```python
from build123d import *

# Parameters (mm, degrees)
SKETCH_1_W                   = 50
SKETCH_1_H                   = 120
EXTRUDE_1_DEPTH              = 6
HOLE_WIZARD_M4_1_D           = 4.5
HOLE_WIZARD_M4_1_CBORE_D     = 8
HOLE_WIZARD_M4_1_CBORE_DEPTH = 4.6
HOLE_WIZARD_M5_3_D           = 5.5
HOLE_WIZARD_M5_3_CBORE_D     = 9.5
HOLE_WIZARD_M5_3_CBORE_DEPTH = 5.7
HOLE_WIZARD_M6_1_D           = 5
HOLE_WIZARD_M6_1_DEPTH       = 15
HOLE_WIZARD_M6_1_TIP         = 1.502151548
HOLE_WIZARD_M5_1_D           = 5.5
HOLE_WIZARD_M5_1_CBORE_D     = 10
HOLE_WIZARD_M5_1_CBORE_DEPTH = 5.7
CHAMFER_1_SIZE               = 1
HOLE_WIZARD_M5_4_D           = 5.5
HOLE_WIZARD_M5_4_CBORE_D     = 10
HOLE_WIZARD_M5_4_CBORE_DEPTH = 5.7


with BuildPart() as part:
    # 草图1 → 凸台-拉伸1 (new, symmetric)
    with BuildSketch(Plane(origin=(0, 0, 0), x_dir=(1, 0, 0), z_dir=(0, 1, 0))):
        Rectangle(SKETCH_1_W, SKETCH_1_H)
    extrude(amount=EXTRUDE_1_DEPTH, both=True)

    # M4 六角圆柱头螺钉的柱形沉头孔1 (through all)
    with Locations(Plane(origin=(0, 6, 0), x_dir=(1, 0, 0), z_dir=(0, 1, 0))):
        with Locations((2, 15), (-20, 30), (2, 30), (-20, 15), (-20, -15), (2, -30), (-20, -30), (2, -15)):
            CounterBoreHole(HOLE_WIZARD_M4_1_D / 2, HOLE_WIZARD_M4_1_CBORE_D / 2, HOLE_WIZARD_M4_1_CBORE_DEPTH)

    # M5 六角圆柱头螺钉的柱形沉头孔3 (through all)
    with Locations(Plane(origin=(0, -6, 0), x_dir=(-1, 0, 0), z_dir=(0, -1, 0))):
        with Locations((16.499999999, -55), (1.500000001, -55), (1.500000001, 55), (16.499999999, 55)):
            CounterBoreHole(HOLE_WIZARD_M5_3_D / 2, HOLE_WIZARD_M5_3_CBORE_D / 2, HOLE_WIZARD_M5_3_CBORE_DEPTH)

    # M6 螺纹孔1
    with Locations(Plane(origin=(0, 6, 0), x_dir=(1, 0, 0), z_dir=(0, 1, 0))):
        with Locations((-9, 10), (-9, -10)):
            Hole(HOLE_WIZARD_M6_1_D / 2, depth=HOLE_WIZARD_M6_1_DEPTH)
            with Locations((0, 0, -(HOLE_WIZARD_M6_1_DEPTH + HOLE_WIZARD_M6_1_TIP / 2))):  # 118° drill point
                Cone(0, HOLE_WIZARD_M6_1_D / 2, HOLE_WIZARD_M6_1_TIP, mode=Mode.SUBTRACT)

    # M5 六角圆柱头螺钉的柱形沉头孔1 (through all)
    with Locations(Plane(origin=(0, 6, 0), x_dir=(1, 0, 0), z_dir=(0, 1, 0))):
        with Locations((1, 40), (1, -40), (-19, -40), (-19, 40)):
            CounterBoreHole(HOLE_WIZARD_M5_1_D / 2, HOLE_WIZARD_M5_1_CBORE_D / 2, HOLE_WIZARD_M5_1_CBORE_DEPTH)

    # 倒角1
    chamfer_1_edges = [part.edges().sort_by_distance(p)[0] for p in [
        (25, 0, 60),
        (-25, 0, 60),
        (-25, 0, -60),
        (25, 0, -60),
    ]]
    chamfer(chamfer_1_edges, length=CHAMFER_1_SIZE)

    # M5 六角圆柱头螺钉的柱形沉头孔4 (through all)
    with Locations(Plane(origin=(0, -6, 0), x_dir=(-1, 0, 0), z_dir=(0, -1, 0))):
        with Locations((-14.5, 50), (-14.5, 0), (-14.5, -50)):
            CounterBoreHole(HOLE_WIZARD_M5_4_D / 2, HOLE_WIZARD_M5_4_CBORE_D / 2, HOLE_WIZARD_M5_4_CBORE_DEPTH)


solid = part.part
```
CAD build for the part. Positions are in the model's coordinates, mm. A direction names the side the tool comes from. Coordinates: 2 decimals unless noted, no trailing zeros. Order: outer loops, then holes, each group sorted by start corner. A loop starts at its lowest first (then second) coordinate and runs counter-clockwise, first axis right, second up. Notation, with made-up numbers: M -39.75,66.5 L -20.75,66.5 A9 cw -20.75,83.5 Z; hole C 3.5,-28 d10. An arc over 180 degrees is marked long. Write each question's results on one line, items separated by ' | '. Start each with the question number.
Q1. Cut at A-A (x = 14.5). List the corners of the cut face in (y, z), then the cut area to 3 significant figures.
Q2. Which spindle directions (+Z, -Z, +X, -X, +Y, -Y) get a long thin tool onto all of the face, cutting with end or side? Do faces 1 (the flat face through (12, -0.3, -48)), 2 (the flat face through (4, 1.4, 32)), 3 (the cylindrical face through (0.79, -2.352, -31.897)). Say none if no direction does.
Q3. Pull direction Z, two halves, no side cores. Call faces 4 (the flat face through (0, 0, -60)), 5 (the flat face through (25, 0, 1)), 6 (the flat face through (-4, -0.3, 57)): +Z half, -Z half, draft (parallel to the pull), parting line (faces both ways), or undercut.
Q4. Drill centre lines: probe 1 along X at (y, z) = (2.25, -40); probe 2 along X at (y, z) = (-4.5, -40); probe 3 along X at (y, z) = (1.75, 50). Where is each one in solid material? Low to high. Write a range as from..to.
Q5. Cut at C-C (y = -3). Count the separate pieces of the cut face and the enclosed holes in it, then the cut area to 3 significant figures.
Q6. Cut at D-D (z = -15). List the corners of the cut face in (x, y).
Q7. Cut at B-B (z = 0). List the corners of the cut face in (x, y), then the cut area to 3 significant figures.
Q8. Flat gauge pins, fed straight in: P1, Ø7, axis at x = -16.5, z = 55, coming from the -Y side; P2, Ø2.5, axis at x = -19, z = -13, coming from the +Y side; P3, Ø5, axis at x = 2, z = -38, coming from the +Y side; P4, Ø4.5, axis at x = -16.5, z = -55, coming from the +Y side. Where does each tip first touch, or does it go through?
Found:
1) outline: M -6,-60 L 6,-60 L 6,-52.75 L -0.3,-52.75 L -0.3,-55 L -6,-55 Z; M -6,-45 L -0.3,-45 L -0.3,-47.25 L 6,-47.25 L 6,-2.75 L -0.3,-2.75 L -0.3,-5 L -6,-5 Z; M -6,5 L -0.3,5 L -0.3,2.75 L 6,2.75 L 6,47.25 L -0.3,47.25 L -0.3,45 L -6,45 Z; M -6,55 L -0.3,55 L -0.3,52.75 L 6,52.75 L 6,60 L -6,60 Z | area: 1,170 mm²
2) face 1: -Y | face 2: +Y | face 3: +Y, -Y
3) face 4: -Z half | face 5: draft | face 6: undercut
4) probe 1: -25..-24, -14..-4, 6..25 | probe 2: -25..-21.75, -16.25..-1.75, 3.75..25 | probe 3: -25..11.75, 17.25..25
5) separate pieces: 1 | enclosed holes: 21 | area: 5,220 mm²
6) outline: M -25,-6 L -22.25,-6 L -22.25,1.4 L -24,1.4 L -24,6 L -25,6 Z; M -17.75,-6 L -0.25,-6 L -0.25,1.4 L -2,1.4 L -2,6 L -16,6 L -16,1.4 L -17.75,1.4 Z; M 4.25,-6 L 25,-6 L 25,6 L 6,6 L 6,1.4 L 4.25,1.4 Z
7) outline: M -25,-6 L 9.5,-6 L 9.5,-0.3 L 11.75,-0.3 L 11.75,6 L -25,6 Z; M 17.25,-0.3 L 19.5,-0.3 L 19.5,-6 L 25,-6 L 25,6 L 17.25,6 Z | area: 508 mm²
8) P1: y = -0.3 | P2: y = 1.4 | P3: y = 0.3 | P4: through
